Here's how the part is built. I have some questions about the finished solid (model axes, mm). Face numbers are marked on the shaded views. A direction names the side the tool comes from. Give positions to 0.01 mm unless a question says otherwise; leave off trailing zeros. Write each loop counter-clockwise with the first axis right and the second up, starting at its lowest first coordinate (ties: lowest second). Pieces come first, ordered by that corner, then holes. Notation, with made-up numbers: (49, 11.5) - (75, 11.5) arc R25 ccw to (75, 43.5) - close; hole circle Ø8 at (21.5, 32). An arc over 180 degrees is marked (long way). Write each question's results on one line, items separated by ' | '. Start each with the question number.
Item 1: Suppose I cut it at B-B on x = 118.5. List the corners of the cut face in (y, z) for me, then the cut area to 3 significant figures.
Item 2: Suppose I cut it at A-A on y = -2.75. List the corners of the cut face in (x, z) for me, then the cut area to 3 significant figures.
Item 3: Please list where these lines run through material, in increasing order: line 1 along X through (y, z) = (-4.5, -27); line 2 along Z through (x, y) = (46.5, 2); line 3 along Z through (x, y) = (127, 3.25).
Item 4: Will these pins go through, and if not, where does the flat tip stop? P1, Ø5, axis at x = 145.5, y = 0, coming from the +Z side; P2, Ø2, axis at x = 116, y = -0.5, coming from the -Z side; P3, Ø3, axis at x = 5, y = -2, coming from the -Z side; P4, Ø4, axis at y = 1, z = -20, coming from the -X side.
Item 5: Suppose I cut it at C-C on z = -32. List the corners of the cut face in (x, y) for me, then the cut area to 3 significant figures.
Item 6: Which directions (+Z, -Z, +X, -X, +Y, -Y) give clear straight access to the entire face, cutting with the end or side of a thin tool? Please do the marked faces 4, 5 and 6.
Item 7: We'd pull the mould along Z, two halves only. Please class the marked faces 1, 2 and 3: +Z half, -Z half, draft (parallel to the pull), parting line (faces both ways), or undercut.
Item 8: Suppose I cut it at D-D on y = 3.25. List the corners of the cut face in (x, z) for me.
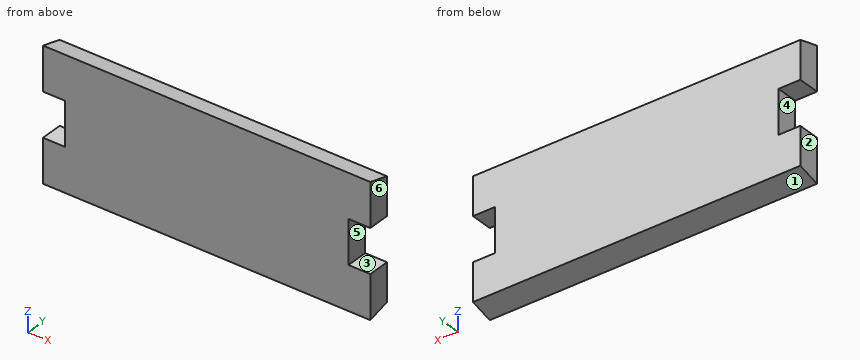
```python
from build123d import *

# Parameters (mm, degrees)
TOP_PLATE_150X60X10_DEPTH = 5
FACE_DRAFT_15_A_ANGLE     = -15
FACE_DRAFT_15_B_ANGLE     = -15


with BuildPart() as part:
    # Top Plate Profile → Top Plate 150x60x10 (new, symmetric)
    with BuildSketch(Plane(origin=(0, 0, 0), x_dir=(1, 0, 0), z_dir=(0, 1, 0))):
        Polygon((0, 0), (150, 0), (150, 20), (140, 20), (140, 40), (150, 40), (150, 60), (0, 60), (0, 40), (10, 40), (10, 20), (0, 20), align=None)
    extrude(amount=TOP_PLATE_150X60X10_DEPTH, both=True)

    # Face Draft 15° A
    face_draft_15_a_faces = [part.faces().sort_by_distance(p)[0] for p in [
        (75, 0, 0),
    ]]
    draft(face_draft_15_a_faces, Plane(origin=(0, -5, 0), x_dir=(0, 0, -1), z_dir=(0, -1, 0)), FACE_DRAFT_15_A_ANGLE)

    # Face Draft 15° B
    face_draft_15_b_faces = [part.faces().sort_by_distance(p)[0] for p in [
        (75, 0, -60),
    ]]
    draft(face_draft_15_b_faces, Plane(origin=(0, -5, 0), x_dir=(0, 0, -1), z_dir=(0, -1, 0)), FACE_DRAFT_15_B_ANGLE)


solid = part.part
```
Checked values:
1) outline: (-5, -60) - (5, -57.32) - (5, -2.68) - (-5, 0) - close | area: 573 mm^2
2) outline: (0, -59.4) - (150, -59.4) - (150, -40) - (140, -40) - (140, -20) - (150, -20) - (150, -0.6) - (0, -0.6) - (0, -20) - (10, -20) - (10, -40) - (0, -40) - close | area: 8,420 mm^2
3) line 1: x = 10 to 140 | line 2: z = -58.12 to -1.88 | line 3: z = -57.79 to -2.21
4) P1: stops at z = -0.67 | P2: stops at z = -59.06 | P3: stops at z = -59.6 | P4: stops at x = 0
5) outline: (10, -5) - (140, -5) - (140, 5) - (10, 5) - close | area: 1,300 mm^2
6) face 4: -X, +Y, -Y | face 5: +X, +Y, -Y | face 6: +Z, -Z, +X, +Y, -Y
7) face 1: -Z half | face 2: draft | face 3: undercut
8) outline: (0, -57.79) - (150, -57.79) - (150, -40) - (140, -40) - (140, -20) - (150, -20) - (150, -2.21) - (0, -2.21) - (0, -20) - (10, -20) - (10, -40) - (0, -40) - close
